Part model, mm, in its own coordinate system. Face numbers are marked on the shaded views. Round coordinates to 2 decimals unless told otherwise and drop trailing zeros. Write each loop counter-clockwise with the first axis right and the second up, starting at its lowest first coordinate (ties: lowest second). Pieces come first, ordered by that corner, then holes.
```python
from build123d import *

# Parameters (mm, degrees)
SKETCH1_R           = 7.5
SKETCH1_R_2         = 4.75
BOSS_EXTRUDE1_DEPTH = 20
SKETCH2_R           = 6
CUT_EXTRUDE1_DEPTH  = 3
SKETCH3_OUTSIDE_W   = 22.83
SKETCH3_OUTSIDE_H   = 22.83
SKETCH3_OUTSIDE_R   = 6.5
CUT_EXTRUDE2_DEPTH  = 15
CHAMFER1_SIZE       = 0.6
CHAMFER1_SIZE2      = 10
CHAMFER2_SIZE       = 0.3
CHAMFER3_SIZE       = 4
CHAMFER3_SIZE2      = 1


with BuildPart() as part:
    # Sketch1 → Boss-Extrude1 (new body)
    with BuildSketch(Plane(origin=(0, 0, 0), x_dir=(1, 0, 0), z_dir=(0, 1, 0))):
        with Locations(Location((0, 0, 0), (0, 0, 270))):
            Circle(SKETCH1_R)
        with Locations(Location((0, 0, 0), (0, 0, 270))):
            Circle(SKETCH1_R_2, mode=Mode.SUBTRACT)
    extrude(amount=BOSS_EXTRUDE1_DEPTH)

    # Sketch2 → Cut-Extrude1 (cut)
    with BuildSketch(Plane(origin=(0, 20, 0), x_dir=(1, 0, 0), z_dir=(0, 1, 0))):
        with Locations(Location((0, 0, 0), (0, 0, 270))):
            Circle(SKETCH2_R)
    extrude(amount=-CUT_EXTRUDE1_DEPTH, mode=Mode.SUBTRACT)

    # Sketch3 outside → Cut-Extrude2 (cut)
    with BuildSketch(Plane.XZ):
        Rectangle(SKETCH3_OUTSIDE_W, SKETCH3_OUTSIDE_H)
        with Locations(Location((0, 0, 0), (0, 0, 270))):
            Circle(SKETCH3_OUTSIDE_R, mode=Mode.SUBTRACT)
    extrude(amount=-CUT_EXTRUDE2_DEPTH, mode=Mode.SUBTRACT)

    # Chamfer1
    chamfer1_edges = [part.edges().sort_by_distance(p)[0] for p in [
        (0, 17, -4.75),
    ]]
    chamfer1_side = [part.faces().sort_by_distance(p)[0] for p in [
        (0, 17, -5.830294373),
    ]]
    chamfer(chamfer1_edges, length=CHAMFER1_SIZE, length2=CHAMFER1_SIZE2, reference=chamfer1_side[0])

    # Chamfer2
    chamfer2_edges = [part.edges().sort_by_distance(p)[0] for p in [
        (0, 15, -7.5),
    ]]
    chamfer(chamfer2_edges, length=CHAMFER2_SIZE)

    # Chamfer3
    chamfer3_edges = [part.edges().sort_by_distance(p)[0] for p in [
        (0, 0, 6.5),
    ]]
    chamfer3_side = [part.faces().sort_by_distance(p)[0] for p in [
        (0, 7.5, 6.5),
    ]]
    chamfer(chamfer3_edges, length=CHAMFER3_SIZE, length2=CHAMFER3_SIZE2, reference=chamfer3_side[0])


solid = part.part
```
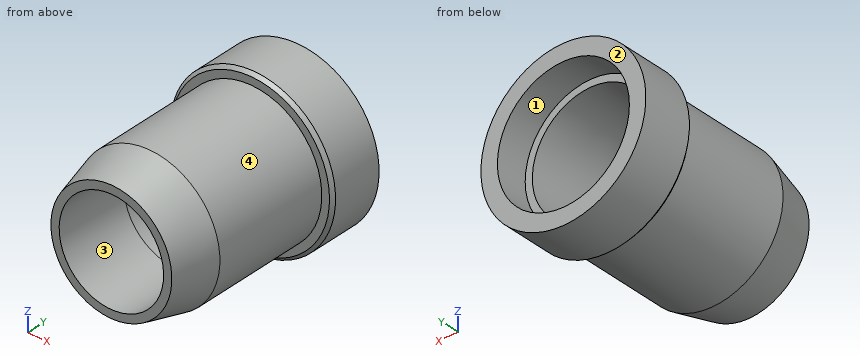
Q1. Cut at A-A on x = 0. Write the cut outline in (y, z).
Values follow:
outline: (0, -5.5) - (4, -6.5) - (15, -6.5) - (15, -7.2) - (15.3, -7.5) - (20, -7.5) - (20, -6) - (17, -6) - (17, -5.35) - (7, -4.75) - (0, -4.75) - close; (0, 4.75) - (7, 4.75) - (17, 5.35) - (17, 6) - (20, 6) - (20, 7.5) - (15.3, 7.5) - (15, 7.2) - (15, 6.5) - (4, 6.5) - (0, 5.5) - close
Q2. Cut at D-D on y = 5.25. Write the cut outline in (x, z).
Values follow:
outline: circle Ø13 at (0, 0); hole circle Ø9.5 at (0, 0)
Q3. Drop flat-ended pins along their axis: pin 1 (4 mm diameter, centred on y = 9.5, z = 4, fed in from +X); pin 2 (2 mm diameter, centred on x = -4, y = 10, fed in from -Z); pin 3 (2 mm diameter, centred on y = 11, z = -4, fed in from +X). Give the stop position or say it passes through.
Values follow:
pin 1: stops at x = 6.18
pin 2: stops at z = -5.77
pin 3: stops at x = 5.77
Q4. Mould opens along X. For the marked faces 1, 2, 3 and 4 say: +X half, -X half, draft (parallel to the pull), parting line (faces both ways), or undercut.
Values follow:
face 1: undercut
face 2: draft
face 3: undercut
face 4: parting line
Q5. Wall check: L1, parallel to Z at x = -0.25, y = 17.75; L2, parallel to X at y = 19.45, z = 0; L3, parallel to Z at x = 0, y = 2.5 (3 decimals). Give the ranges that are in metal, low to high.
Values follow:
L1: z = -7.5 to -5.99, 5.99 to 7.5
L2: x = -7.5 to -6, 6 to 7.5
L3: z = -6.125 to -4.75, 4.75 to 6.125
Q6. Cut at B-B on z = 0. Write the cut outline in (x, y).
Values follow:
outline: (-7.5, 15.3) - (-7.2, 15) - (-6.5, 15) - (-6.5, 4) - (-5.5, 0) - (-4.75, 0) - (-4.75, 7) - (-5.35, 17) - (-6, 17) - (-6, 20) - (-7.5, 20) - close; (4.75, 0) - (5.5, 0) - (6.5, 4) - (6.5, 15) - (7.2, 15) - (7.5, 15.3) - (7.5, 20) - (6, 20) - (6, 17) - (5.35, 17) - (4.75, 7) - close
Q7. Cut at C-C on y = 10. Write the cut outline in (x, z).
Values follow:
outline: circle Ø13 at (0, 0); hole circle Ø9.86 at (0, 0)
